Model file for the job. Use its own axes, mm. Coordinates: 2 decimals unless noted, no trailing zeros. Return JSON: item names as keys, results as strings.
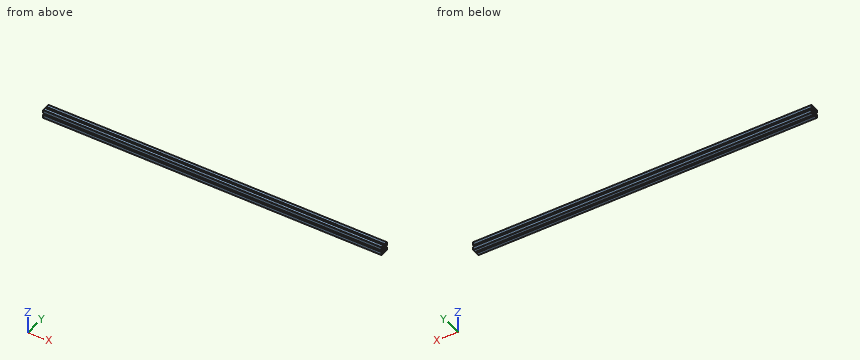
```python
from build123d import *

# Parameters (mm, degrees)
SKETCH_11_R         = 3
SKETCH_11_R_2       = 2.5
F_0_GY_3030_1_DEPTH = 1200


with BuildPart() as part:
    # 草图11 → 0国耀铝型材 GY-3030国标铝型材(1) (new body)
    with BuildSketch(Plane.YZ):
        with BuildLine():
            Line((-14, -15), (-3.15, -15))
            Line((-3.15, -15), (-3.15, -12.5))
            Line((-3.15, -12.5), (-5.15, -12.5))
            Line((-5.15, -12.5), (-5.15, -6.5))
            ThreePointArc((-5.15, -6.5), (-3.019390742, -5.122695475), (-0.555, -4.52))
            Line((-0.555, -4.52), (0, -4.2))
            Line((0, -4.2), (0.555, -4.52))
            ThreePointArc((0.555, -4.52), (3.019390742, -5.122695475), (5.15, -6.5))
            Line((5.15, -6.5), (5.15, -12.5))
            Line((5.15, -12.5), (3.15, -12.5))
            Line((3.15, -12.5), (3.15, -15))
            Line((3.15, -15), (14, -15))
            ThreePointArc((14, -15), (14.707106781, -14.707106781), (15, -14))
            Line((15, -14), (15, -3.15))
            Line((15, -3.15), (12.5, -3.15))
            Line((12.5, -3.15), (12.5, -5.15))
            Line((12.5, -5.15), (6.5, -5.15))
            ThreePointArc((6.5, -5.15), (5.12253592, -3.018923167), (4.52, -0.554))
            Line((4.52, -0.554), (4.2, 0))
            Line((4.2, 0), (4.52, 0.555))
            ThreePointArc((4.52, 0.555), (5.122695475, 3.019390742), (6.5, 5.15))
            Line((6.5, 5.15), (12.5, 5.15))
            Line((12.5, 5.15), (12.5, 3.15))
            Line((12.5, 3.15), (15, 3.15))
            Line((15, 3.15), (15, 14))
            ThreePointArc((15, 14), (14.707106781, 14.707106781), (14, 15))
            Line((14, 15), (3.15, 15))
            Line((3.15, 15), (3.15, 12.5))
            Line((3.15, 12.5), (5.15, 12.5))
            Line((5.15, 12.5), (5.15, 6.5))
            ThreePointArc((5.15, 6.5), (3.019292492, 5.123227892), (0.555, 4.521))
            Line((0.555, 4.521), (0, 4.2))
            Line((0, 4.2), (-0.555, 4.521))
            ThreePointArc((-0.555, 4.521), (-3.019292492, 5.123227892), (-5.15, 6.5))
            Line((-5.15, 6.5), (-5.15, 12.5))
            Line((-5.15, 12.5), (-3.15, 12.5))
            Line((-3.15, 12.5), (-3.15, 15))
            Line((-3.15, 15), (-14, 15))
            ThreePointArc((-14, 15), (-14.707106781, 14.707106781), (-15, 14))
            Line((-15, 14), (-15, 3.15))
            Line((-15, 3.15), (-12.5, 3.15))
            Line((-12.5, 3.15), (-12.5, 5.15))
            Line((-12.5, 5.15), (-6.5, 5.15))
            ThreePointArc((-6.5, 5.15), (-5.122695475, 3.019390742), (-4.52, 0.555))
            Line((-4.52, 0.555), (-4.2, 0))
            Line((-4.2, 0), (-4.52, -0.554))
            ThreePointArc((-4.52, -0.554), (-5.12253592, -3.018923167), (-6.5, -5.15))
            Line((-6.5, -5.15), (-12.5, -5.15))
            Line((-12.5, -5.15), (-12.5, -3.15))
            Line((-12.5, -3.15), (-15, -3.15))
            Line((-15, -3.15), (-15, -14))
            ThreePointArc((-15, -14), (-14.707106781, -14.707106781), (-14, -15))
        make_face()
        with Locations((9.8, 9.9)):
            Circle(SKETCH_11_R, mode=Mode.SUBTRACT)
        with Locations((9.8, -9.9)):
            Circle(SKETCH_11_R, mode=Mode.SUBTRACT)
        Circle(SKETCH_11_R_2, mode=Mode.SUBTRACT)
        with Locations((-9.8, 9.9)):
            Circle(SKETCH_11_R, mode=Mode.SUBTRACT)
        with Locations((-10, -9.9)):
            Circle(SKETCH_11_R, mode=Mode.SUBTRACT)
    extrude(amount=F_0_GY_3030_1_DEPTH)


solid = part.part
```
Item 1: Wall check: line 1 (Z direction, x = 503, y = 9.8); line 2 (Y direction, x = 927.5, z = -9.5); line 3 (Y direction, x = 1017, z = -13). Give the ranges that are in metal, low to high.
Check result:
{"line 1": "z = -15 to -12.9, -6.9 to -5.15, 5.15 to 6.9, 12.9 to 15", "line 2": "y = -15 to -12.97, -7.03 to -5.15, 5.15 to 6.83, 12.77 to 15", "line 3": "y = -15 to -3.15, 3.15 to 15"}
Item 2: Drop a flat-ended pin along its axis: pin 1 Ø1.5 at (y, z) = (-3.5, -10.5) entering from +X. Give the stop position or say it passes through.
Check result:
{"pin 1": "passes through"}
Item 3: Saw through at A-A (x = 238.5). Count the separate pieces of the cut face and the enclosed holes in it, and give its area (3 significant figures).
Check result:
{"separate pieces": "1", "enclosed holes": "5", "area": "399 mm2"}
